```python
from build123d import *

# Parameters (mm, degrees)
END_LOOPS_DEPTH       = 25
END_LOOPS_2_DEPTH     = 25
CENTRE_BLOCK_SKETCH_W = 80
CENTRE_BLOCK_SKETCH_H = 40
CENTRE_BLOCK_DEPTH    = 20
CROSS_HOLE_SKETCH_R   = 4.957337167
CROSS_HOLE_DEPTH      = 164


with BuildPart() as part:
    # End Loops Sketch → End Loops (new, symmetric)
    with BuildSketch(Plane.XY):
        with BuildLine():
            Line((-40, 35), (-40, -25))
            ThreePointArc((-40, -25), (-55, -40), (-70, -25))
            Line((-70, -25), (-70, 35))
            ThreePointArc((-70, 35), (-55, 50), (-40, 35))
        make_face()
        with BuildLine():
            Line((-45, 35), (-45, -25))
            ThreePointArc((-45, -25), (-55, -35), (-65, -25))
            Line((-65, -25), (-65, 35))
            ThreePointArc((-65, 35), (-55, 45), (-45, 35))
        make_face(mode=Mode.SUBTRACT)
    extrude(amount=END_LOOPS_DEPTH, both=True)



with BuildPart() as body_2:
    # End Loops Sketch → End Loops 2 (new, symmetric)
    with BuildSketch(Plane.XY):
        with BuildLine():
            Line((70, 35), (70, -25))
            ThreePointArc((70, -25), (55, -40), (40, -25))
            Line((40, -25), (40, 35))
            ThreePointArc((40, 35), (55, 50), (70, 35))
        make_face()
        with BuildLine():
            Line((65, 35), (65, -25))
            ThreePointArc((65, -25), (55, -35), (45, -25))
            Line((45, -25), (45, 35))
            ThreePointArc((45, 35), (55, 45), (65, 35))
        make_face(mode=Mode.SUBTRACT)
    extrude(amount=END_LOOPS_2_DEPTH, both=True)


with BuildPart() as part_1:
    add(part.part)

    add(body_2.part)  # Centre Block merges body 2
    # Centre Block Sketch → Centre Block (add, symmetric)
    with BuildSketch(Plane.XY):
        with Locations((0, 5)):
            Rectangle(CENTRE_BLOCK_SKETCH_W, CENTRE_BLOCK_SKETCH_H)
        with BuildLine():
            Line((-20, 15), (20, 15))
            ThreePointArc((20, 15), (30, 5), (20, -5))
            Line((20, -5), (-20, -5))
            ThreePointArc((-20, -5), (-30, 5), (-20, 15))
        make_face(mode=Mode.SUBTRACT)
    extrude(amount=CENTRE_BLOCK_DEPTH, both=True)

    # Cross Hole Sketch → Cross Hole (cut)
    with BuildSketch(Plane(origin=(70, 0, 0), x_dir=(0, 0, -1), z_dir=(1, 0, 0))):
        with Locations(Location((0, 5, 0), (0, 0, 90))):
            Circle(CROSS_HOLE_SKETCH_R)
    extrude(amount=-CROSS_HOLE_DEPTH, mode=Mode.SUBTRACT)


solid = part_1.part
```
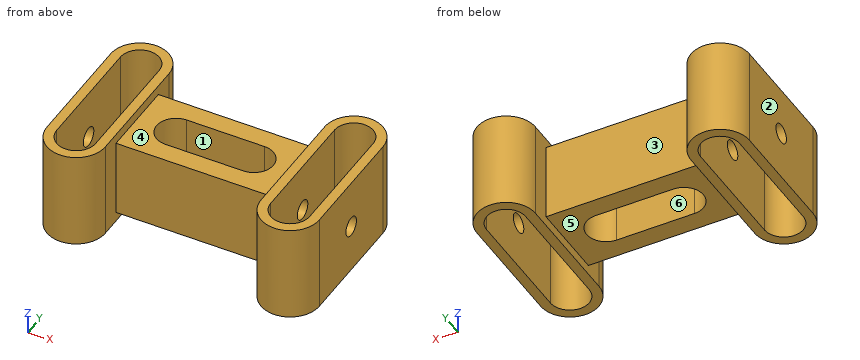
Verification items for the finished model (mm, model axes). Face numbers are marked on the shaded views. A direction names the side the tool comes from. Coordinates: 2 decimals unless noted, no trailing zeros. Order: outer loops, then holes, each group sorted by start corner. A loop starts at its lowest first (then second) coordinate and runs counter-clockwise, first axis right, second up. Notation, with made-up numbers: (-39.75, 38.25) - (-26.75, 38.25) arc R24 ccw to (-26.75, 57.25) - close; hole circle Ø9 at (88, 13). An arc over 180 degrees is marked (long way). Return JSON: item names as keys, results as strings.
(1) Mould release check, pull along X, two halves, no side actions. Record for the marked faces 1 and 2: pulls with the +X half, pulls with the -X half, needs draft (parallel to the pull), parting line crosses it, or undercut.
Filled sheet:
{"face 1": "undercut", "face 2": "pulls with the -X half"}
(2) Thickness scan on line 1 along X through (y, z) = (29.5, 20.5); line 2 along X through (y, z) = (-6, -2); line 3 along X through (y, z) = (10, 0.5). Record the ranges inside material, lowest first.
Filled sheet:
{"line 1": "x = -70 to -65, -45 to -40, 40 to 45, 65 to 70", "line 2": "x = -70 to -65, -45 to 45, 65 to 70", "line 3": "x = -70 to -65, -45 to -28.66, 28.66 to 45, 65 to 70"}
(3) Section check C-C, the plane z = -8.5. Record the cut outline in (x, y).
Filled sheet:
{"outline": "(-70, -25) arc R15 ccw to (-40, -25) - (-40, -15) - (40, -15) - (40, -25) arc R15 ccw to (70, -25) - (70, 35) arc R15 ccw to (40, 35) - (40, 25) - (-40, 25) - (-40, 35) arc R15 ccw to (-70, 35) - close; hole (-65, -25) arc R10 ccw to (-45, -25) - (-45, 35) arc R10 ccw to (-65, 35) - close; hole (-20, -5) - (20, -5) arc R10 ccw to (20, 15) - (-20, 15) arc R10 ccw to start; hole (45, -25) arc R10 ccw to (65, -25) - (65, 35) arc R10 ccw to (45, 35) - close"}
(4) Section check D-D, the plane y = -23.5. Record the cut outline in (x, z), and give its area (3 significant figures).
Filled sheet:
{"outline": "(-70, -25) - (-65, -25) - (-65, 25) - (-70, 25) - close; (-45, -25) - (-40, -25) - (-40, 25) - (-45, 25) - close; (40, -25) - (45, -25) - (45, 25) - (40, 25) - close; (65, -25) - (70, -25) - (70, 25) - (65, 25) - close", "area": "1,000 mm^2"}
(5) Access from +Z, -Z, +X, -X, +Y, -Y to the whole of each face (thin tool, end or side, straight path). Record for the marked faces 3, 4, 5 and 6.
Filled sheet:
{"face 3": "+Z, -Z, +Y", "face 4": "+Z, +Y, -Y", "face 5": "-Z, +Y, -Y", "face 6": "+Z, -Z"}
(6) Section check A-A, the plane y = -6.5. Record the cut outline in (x, z).
Filled sheet:
{"outline": "(-70, -25) - (-65, -25) - (-65, 25) - (-70, 25) - close; (-45, -25) - (-40, -25) - (-40, -20) - (40, -20) - (40, -25) - (45, -25) - (45, 25) - (40, 25) - (40, 20) - (-40, 20) - (-40, 25) - (-45, 25) - close; (65, -25) - (70, -25) - (70, 25) - (65, 25) - close"}
(7) Go/stop test with flat-tipped pins: pin 1 (12 mm diameter, centred on x = 8, z = -4, fed in from +Y); pin 2 (12 mm diameter, centred on x = -28, y = 3, fed in from +Z); pin 3 (6 mm diameter, centred on x = 47.5, z = -1.5, fed in from +Y). Record where each tip stops, or that it passes through.
Filled sheet:
{"pin 1": "stops at y = 25", "pin 2": "stops at z = 20", "pin 3": "stops at y = 49.31"}
(8) Section check B-B, the plane x = -55. Record the cut outline in (y, z).
Filled sheet:
{"outline": "(-40, -25) - (-35, -25) - (-35, 25) - (-40, 25) - close; (45, -25) - (50, -25) - (50, 25) - (45, 25) - close"}
